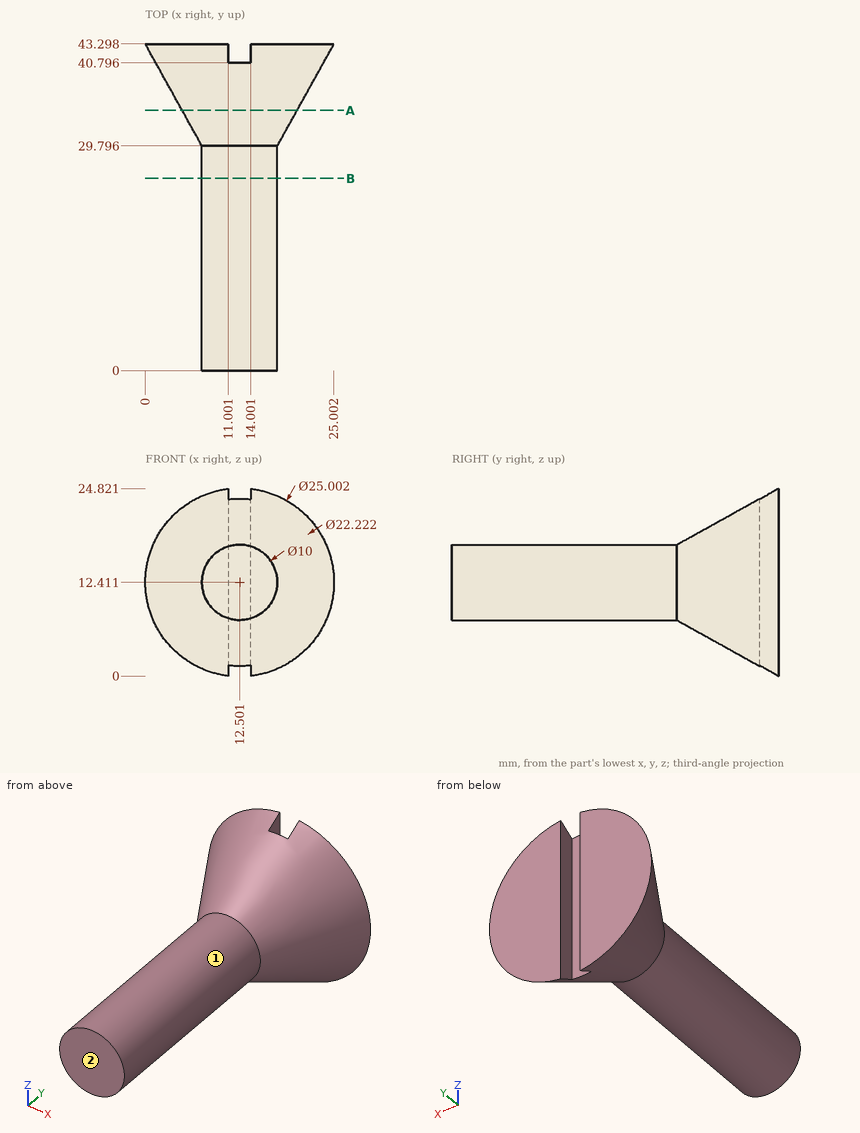
Could you check a few things on this drawing? It's one solid part, dimensions in mm from its lowest x, y, z. A direction names the side the tool comes from. Round coordinates to 2 decimals unless told otherwise and drop trailing zeros. Order: outer loops, then holes, each group sorted by start corner. A loop starts at its lowest first (then second) coordinate and runs counter-clockwise, first axis right, second up. Notation, with made-up numbers: M 42.25,85 L 71.25,85 A9 cw 71.25,97 Z; hole C 3,44.25 d8. An arc over 180 degrees is marked long. One line per item, written item: value.
(1) I'm going to push flat-ended pins straight in: P1, Ø6, axis at x = 7, z = 16, coming from the -Y side; P2, Ø2, axis at x = 10.5, y = 22, coming from the +Z side; P3, Ø12, axis at y = 37, z = 11, coming from the -X side; P4, Ø2.5, axis at x = 12.5, z = 9, coming from the +Y side. Where does each tip first touch, or does it pass through?
Ans:
P1: stops at y = 0
P2: stops at z = 17.31
P3: stops at x = 0.21
P4: stops at y = 40.8
(2) I need wall thicknesses on line 1 along X through (y, z) = (14, 12.25); line 2 along Z through (x, y) = (12.75, 22) (1 decimal); line 3 along Z through (x, y) = (7, 36.5). Which ranges of each line are inside material? Lowest first, please. Write a range as from..to.
Ans:
line 1: x = 7.5..17.5
line 2: z = 7.4..17.4
line 3: z = 5.64..19.18
(3) Imagine slicing it at A-A (y = 34.5). Write out the boundary of the cut face in (x, z), and give its area (3 significant figures).
Ans:
outline: C 12.5,12.41 d15.23
area: 182 mm^2
(4) Which directions (+Z, -Z, +X, -X, +Y, -Y) give clear straight access to the entire face, cutting with the end or side of a thin tool? Please do the marked faces 1 and 2.
Ans:
face 1: -Y
face 2: +Z, -Z, +X, -X, -Y
(5) Imagine slicing it at B-B (y = 25.5). Write out the boundary of the cut face in (x, z).
Ans:
outline: C 12.5,12.41 d10
